Input: part model. Units: mm. Frame: model coordinates. Face numbers are marked on the shaded views. A direction names the side the tool comes from. Round coordinates to 2 decimals unless told otherwise and drop trailing zeros. Order: outer loops, then holes, each group sorted by start corner. A loop starts at its lowest first (then second) coordinate and runs counter-clockwise, first axis right, second up. Notation, with made-up numbers: M -31,77.5 L 25,77.5 A24 ccw 25,95.5 Z; hole C -9,81.25 d7. An arc over 180 degrees is marked long. One line per question, with ' | ' between items.
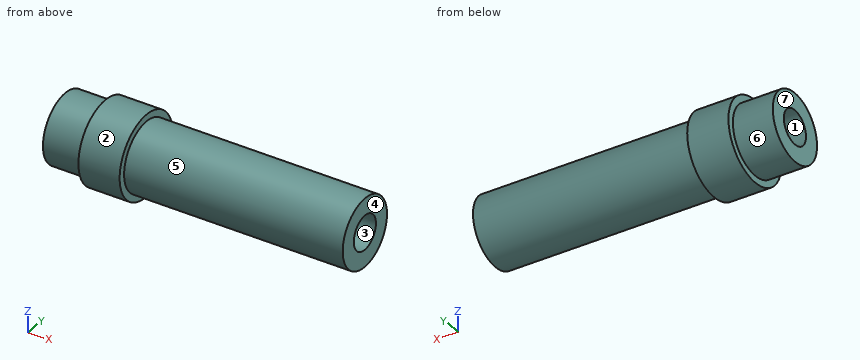
```python
from build123d import *

# Parameters (mm, degrees)
M3_TAPPED_HOLE1_D               = 2.5
M3_TAPPED_HOLE1_DEPTH           = 8
M3_TAPPED_HOLE1_TIP             = 0.751075774
M3_TAPPED_HOLE1_ON_FACE_2_D     = 2.5
M3_TAPPED_HOLE1_ON_FACE_2_DEPTH = 8
M3_TAPPED_HOLE1_ON_FACE_2_TIP   = 0.751075774


with BuildPart() as part:
    # Sketch1 → Revolve1 (revolve)
    with BuildSketch(Plane.XY):
        Polygon((22.305681316, -2.5), (0.505681316, -2.5), (0.505681316, 0), (3.405681316, 0), (3.405681316, 0.5), (6.405681316, 0.5), (6.405681316, 0), (22.305681316, 0), align=None)
    revolve(axis=Axis((22.305681316, -2.5, 0), (-1, 0, 0)))

    # M3 Tapped Hole1
    with Locations(Plane(origin=(0.505681316, -2.5, 0), x_dir=(0, 0, -1), z_dir=(-1, 0, 0))):
        with Locations((0, 0)):
            Hole(M3_TAPPED_HOLE1_D / 2, depth=M3_TAPPED_HOLE1_DEPTH)
            with Locations((0, 0, -(M3_TAPPED_HOLE1_DEPTH + M3_TAPPED_HOLE1_TIP / 2))):  # 118° drill point
                Cone(0, M3_TAPPED_HOLE1_D / 2, M3_TAPPED_HOLE1_TIP, mode=Mode.SUBTRACT)

    # M3 Tapped Hole1 on face 2
    with Locations(Plane(origin=(22.305681316, -2.5, 0), x_dir=(0, 0, 1), z_dir=(1, 0, 0))):
        with Locations((0, 0)):
            Hole(M3_TAPPED_HOLE1_ON_FACE_2_D / 2, depth=M3_TAPPED_HOLE1_ON_FACE_2_DEPTH)
            with Locations((0, 0, -(M3_TAPPED_HOLE1_ON_FACE_2_DEPTH + M3_TAPPED_HOLE1_ON_FACE_2_TIP / 2))):  # 118° drill point
                Cone(0, M3_TAPPED_HOLE1_ON_FACE_2_D / 2, M3_TAPPED_HOLE1_ON_FACE_2_TIP, mode=Mode.SUBTRACT)


solid = part.part
```
Item 1: Section query A-A, the plane x = 20.75. Return loops of the section in (y, z), plus the area to 3 significant figures.
Report:
outline: C -2.5,0 d5; hole C -2.5,0 d2.5 | area: 14.7 mm²
Item 2: First-contact query: pin 1 (2 mm diameter, centred on x = 12, z = 1, fed in from +Y); pin 2 (1.5 mm diameter, centred on x = 4.5, y = -4.5, fed in from -Z); pin 3 (1.5 mm diameter, centred on x = 7.5, y = -3.5, fed in from +Z). Flat tips, straight axial feed; report the tip coordinate or a pass-through.
Report:
pin 1: y = 0 | pin 2: z = -2.73 | pin 3: z = 2.49
Item 3: Mould query, pull axis Z, two halves, no side actions, for the marked faces 1, 2, 3 and 4. Classes: +Z half, -Z half, draft (parallel to the pull), parting line (faces both ways), or undercut.
Report:
face 1: undercut | face 2: parting line | face 3: undercut | face 4: draft
Item 4: Section query C-C, the plane z = -2.1. Return loops of the section in (x, y).
Report:
outline: M 0.51,-3.86 L 3.41,-3.86 L 3.41,-4.64 L 6.41,-4.64 L 6.41,-3.86 L 22.31,-3.86 L 22.31,-1.14 L 6.41,-1.14 L 6.41,-0.36 L 3.41,-0.36 L 3.41,-1.14 L 0.51,-1.14 Z
Item 5: Section query D-D, the plane x = 9.75. Return loops of the section in (y, z).
Report:
outline: C -2.5,0 d5
Item 6: Section query B-B, the plane y = -0.6. Return loops of the section in (x, z), plus the area to 3 significant figures.
Report:
outline: M 0.51,-1.62 L 3.41,-1.62 L 3.41,-2.32 L 6.41,-2.32 L 6.41,-1.62 L 22.31,-1.62 L 22.31,1.62 L 6.41,1.62 L 6.41,2.32 L 3.41,2.32 L 3.41,1.62 L 0.51,1.62 Z | area: 75.0 mm²
Item 7: Line query: line 1 along Y through (x, z) = (16.75, 0); line 2 along X through (y, z) = (-3.7, 2.6); line 3 along Y through (x, z) = (5.75, 0). Output: solid intervals per line, ascending. Write a range as from..to.
Report:
line 1: -5..-3.75, -1.25..0 | line 2: 3.41..6.41 | line 3: -5.5..-3.75, -1.25..0.5
Item 8: Access query for the marked faces 5, 6 and 7. Directions: +Z, -Z, +X, -X, +Y, -Y. A direction counts if a zero-diameter tool reaches every point of the face in a straight line with its end or side. Return the directions, or none.
Report:
face 5: +X | face 6: -X | face 7: +Z, -Z, -X, +Y, -Y
